Input: part model. Units: mm. Frame: model coordinates. Face numbers are marked on the shaded views. A direction names the side the tool comes from. Give positions to 0.01 mm unless a question says otherwise; leave off trailing zeros. Write each loop counter-clockwise with the first axis right and the second up, starting at its lowest first coordinate (ties: lowest second). Pieces come first, ordered by that corner, then holes. Notation, with made-up numbers: (11, -23) - (39, -23) arc R31 ccw to (39, 4) - close; hole circle Ø7 at (51.25, 63). An arc over 180 degrees is marked (long way). Answer as CSV lines item,"result". Start each with the question number.
from build123d import *

# Parameters (mm, degrees)
SKETCH_1_W                     = 62
SKETCH_1_H                     = 75
EXTRUDE_1_DEPTH                = 12.5
HOLE_WIZARD_M6_1_D             = 5
CHAMFER_1_SIZE                 = 3
SKETCH_8_W                     = 30
SKETCH_8_H                     = 75
CUT_EXTRUDE_1_DEPTH            = 10
HOLE_WIZARD_M6_2_D             = 5
HOLE_WIZARD_M6_1_2_D           = 6.6
HOLE_WIZARD_M6_1_2_CBORE_D     = 11
HOLE_WIZARD_M6_1_2_CBORE_DEPTH = 20


with BuildPart() as part:
    # 草图1 → 凸台-拉伸1 (new, symmetric)
    with BuildSketch(Plane.XY):
        Rectangle(SKETCH_1_W, SKETCH_1_H)
    extrude(amount=EXTRUDE_1_DEPTH, both=True)

    # Hole Wizard M6 _1 (through all)
    with Locations(Plane.XY.offset(12.5)):
        with Locations((0, 0)):
            Hole(HOLE_WIZARD_M6_1_D / 2)

    # 倒角1
    chamfer_1_edges = [part.edges().sort_by_distance(p)[0] for p in [
        (-31, 0, -12.5),
        (31, 0, -12.5),
    ]]
    chamfer(chamfer_1_edges, length=CHAMFER_1_SIZE)

    # 草图8 → 切除-拉伸1 (cut)
    with BuildSketch(Plane(origin=(0, 0, -12.5), x_dir=(-1, 0, 0), z_dir=(0, 0, -1))):
        Rectangle(SKETCH_8_W, SKETCH_8_H)
    extrude(amount=-CUT_EXTRUDE_1_DEPTH, mode=Mode.SUBTRACT)

    # M6 螺纹孔2 (through all)
    with Locations(Plane(origin=(0, 0, -2.5), x_dir=(-1, 0, 0), z_dir=(0, 0, -1))):
        with Locations((0, 22.5), (0, -22.5)):
            Hole(HOLE_WIZARD_M6_2_D / 2)

    # Hole Wizard M6 _1 2 (through all)
    with Locations(Plane(origin=(0, 0, -12.5), x_dir=(-1, 0, 0), z_dir=(0, 0, -1))):
        with Locations((-14.5, -3.5), (14.5, -3.5)):
            CounterBoreHole(HOLE_WIZARD_M6_1_2_D / 2, HOLE_WIZARD_M6_1_2_CBORE_D / 2, HOLE_WIZARD_M6_1_2_CBORE_DEPTH)


solid = part.part
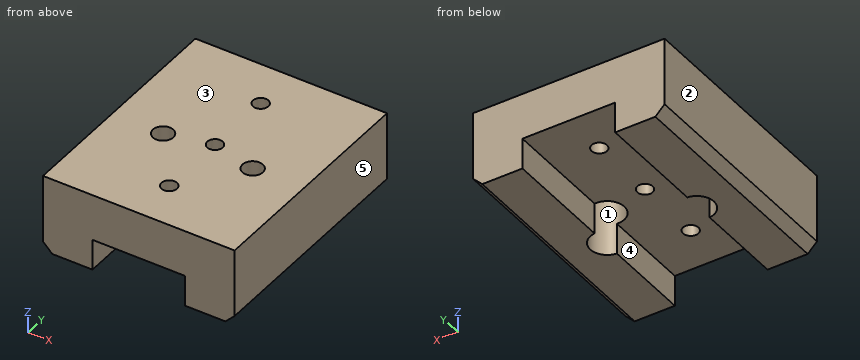
1) Cut plane B-B on y = -3.5. Output: boundary loops of the cut face in (x, z).
2) Cut plane C-C on y = -22.5. Output: boundary loops of the cut face in (x, z), and give its area (3 significant figures).
3) Reachability of the marked faces 4 and 5 from +Z, -Z, +X, -X, +Y, -Y: full face, straight path, thin tool, end or side. Return the list, or none.
4) Cut plane A-A on z = -6.75. Output: boundary loops of the cut face in (x, y), and give its area (3 significant figures).
5) Material intervals for line 1 (X direction, y = -3.5, z = -1.5); line 2 (Y direction, x = 0, z = 5); line 3 (Y direction, x = 14.5, z = 2.5), sorted ascending. Write a range as from..to.
6) Pull-direction query (X, two-part tool) for the marked faces 1, 2 and 3; classes: +X half, -X half, draft (parallel to the pull), parting line (faces both ways), or undercut.
7) Cut plane D-D on z = -1. Output: boundary loops of the cut face in (x, y), and give its area (3 significant figures).
8) Contact query for flat-ended pins moving along their axis: P1, Ø3.5, axis at x = 12.5, y = -1.5, coming from the -Z side; P2, Ø5.5, axis at x = -14.5, y = -3.5, coming from the -Z side; P3, Ø5.5, axis at x = -13, y = -6, coming from the -Z side. Output: stop coordinate, or through.
Numbers:
1,outline,"(-31, -9.5) - (-28, -12.5) - (-20, -12.5) - (-20, 7.5) - (-17.8, 7.5) - (-17.8, 12.5) - (-31, 12.5) - close; (-11.2, 7.5) - (-9, 7.5) - (-9, -2.5) - (9, -2.5) - (9, 7.5) - (11.2, 7.5) - (11.2, 12.5) - (-11.2, 12.5) - close; (17.8, 7.5) - (20, 7.5) - (20, -12.5) - (28, -12.5) - (31, -9.5) - (31, 12.5) - (17.8, 12.5) - close"
2,outline,"(-31, -9.5) - (-28, -12.5) - (-15, -12.5) - (-15, -2.5) - (-2.5, -2.5) - (-2.5, 12.5) - (-31, 12.5) - close; (2.5, -2.5) - (15, -2.5) - (15, -12.5) - (28, -12.5) - (31, -9.5) - (31, 12.5) - (2.5, 12.5) - close"
2,area,"1,170 mm²"
3,face 4,"-Z, +Y, -Y"
3,face 5,"+Z, -Z, +X, +Y, -Y"
4,outline,"(-31, -37.5) - (-15, -37.5) - (-15, -8.98) arc R5.5 cw to (-15, 1.98) - (-15, 37.5) - (-31, 37.5) - close; (15, -37.5) - (31, -37.5) - (31, 37.5) - (15, 37.5) - (15, 1.98) arc R5.5 cw to (15, -8.98) - close"
4,area,"2,320 mm²"
5,line 1,"x = -31..-20, -9..9, 20..31"
5,line 2,"y = -37.5..-25, -20..-2.5, 2.5..20, 25..37.5"
5,line 3,"y = -37.5..-9, 2..37.5"
6,face 1,"undercut"
6,face 2,"-X half"
6,face 3,"draft"
7,outline,"(-31, -37.5) - (31, -37.5) - (31, 37.5) - (-31, 37.5) - close; hole circle Ø11 at (-14.5, -3.5); hole circle Ø5 at (0, -22.5); hole circle Ø5 at (0, 0); hole circle Ø5 at (0, 22.5); hole circle Ø11 at (14.5, -3.5)"
7,area,"4,400 mm²"
8,P1,"stops at z = 7.5"
8,P2,"passes through"
8,P3,"stops at z = -2.5"
